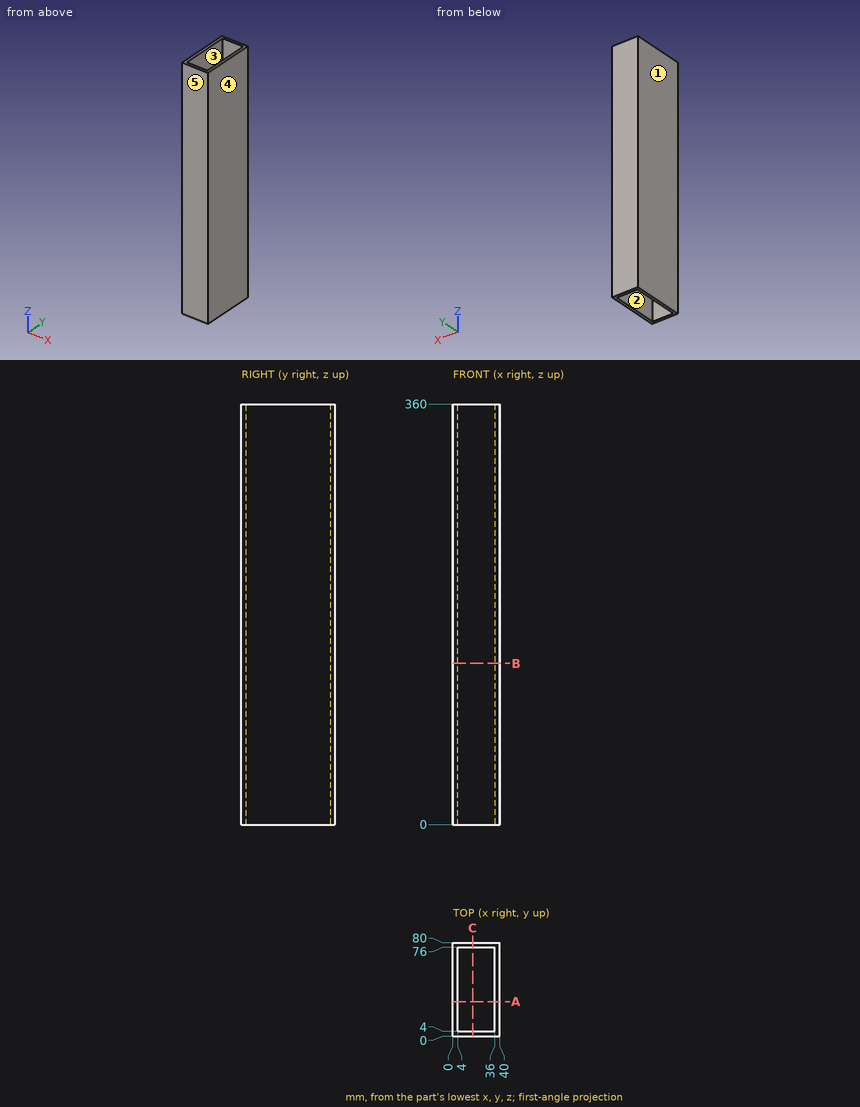
Source: three-view drawing plus pictorial views. Frame: mm from the lowest corner of the part. A direction names the side the tool comes from. Give positions to 0.01 mm unless a question says otherwise; leave off trailing zeros. Order: outer loops, then holes, each group sorted by start corner. A loop starts at its lowest first (then second) coordinate and runs counter-clockwise, first axis right, second up. Notation, with made-up numbers: M -20,-34.75 L 19,-34.75 A27 cw 19,-10.75 Z; hole C 50.25,54.25 d6. An arc over 180 degrees is marked long. One line per question, with ' | ' between items.
1) Ray query, L1, parallel to X at y = 72.5, z = 210; L2, parallel to Y at x = 19, z = 141.5. Return the intervals inside material, ascending.
Filled in:
L1: x = 0 to 4, 36 to 40 | L2: y = 0 to 4, 76 to 80
2) Section A-A on y = 29.5. Output: boundary loops of the cut face in (x, z), and give its area (3 significant figures).
Filled in:
outline: M 0,0 L 4,0 L 4,360 L 0,360 Z; M 36,0 L 40,0 L 40,360 L 36,360 Z | area: 2,880 mm2
3) Draft query along Y for the marked faces 3, 4 and 5. Return one class per face: pulls with the +Y half, pulls with the -Y half, needs draft (parallel to the pull), parting line crosses it, or undercut.
Filled in:
face 3: undercut | face 4: needs draft | face 5: pulls with the -Y half
4) Access query for the marked faces 1 and 2. Directions: +Z, -Z, +X, -X, +Y, -Y. A direction counts if a zero-diameter tool reaches every point of the face in a straight line with its end or side. Return the directions, or none.
Filled in:
face 1: +Z, -Z, -X, +Y, -Y | face 2: +Z, -Z
5) Section C-C on x = 17. Output: boundary loops of the cut face in (y, z).
Filled in:
outline: M 0,0 L 4,0 L 4,360 L 0,360 Z; M 76,0 L 80,0 L 80,360 L 76,360 Z
6) Section B-B on z = 138. Output: boundary loops of the cut face in (x, y).
Filled in:
outline: M 0,0 L 40,0 L 40,80 L 0,80 Z; hole M 4,4 L 36,4 L 36,76 L 4,76 Z
